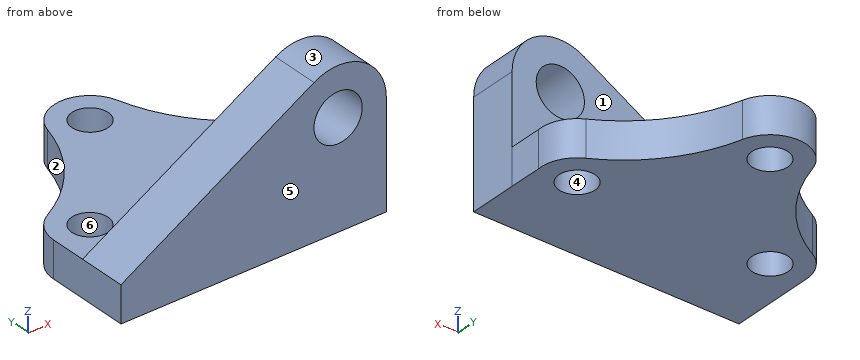
```python
from build123d import *

# Parameters (mm, degrees)
BASE_WEDGE_PROFILE_SKETCH_R     = 10
BASE_WEDGE_BLOCK_DEPTH          = 20
UPRIGHT_FLANGE_PROFILE_SKETCH_R = 7.5
UPRIGHT_FLANGE_PROFILE_SKETCH_W = 110
UPRIGHT_FLANGE_PROFILE_SKETCH_H = 20
UPRIGHT_FLANGE_WITH_HOLES_DEPTH = 15


with BuildPart() as part:
    # Base Wedge Profile Sketch → Base Wedge Block (new body)
    with BuildSketch(Plane(origin=(0, 0, 0), x_dir=(1, 0, 0), z_dir=(0, 1, 0))):
        with BuildLine():
            Line((0, 0), (110, 0))
            Line((110, 0), (110, -28.867513459))
            ThreePointArc((110, -28.867513459), (100, -46.188021535), (80, -46.188021535))
            Line((80, -46.188021535), (0, 0))
        make_face()
        with Locations(Location((90, -28.867513459, 0), (0, 0, 270))):
            Circle(BASE_WEDGE_PROFILE_SKETCH_R, mode=Mode.SUBTRACT)
    extrude(amount=-BASE_WEDGE_BLOCK_DEPTH)

    # Upright Flange Profile Sketch → Upright Flange with Holes (add)
    # profile 1 of 2: a face of its own
    with BuildSketch(Plane(origin=(0, 0, 0), x_dir=(-1, 0, 0), z_dir=(0, 0, -1))):
        with BuildLine():
            ThreePointArc((-40.373259229, 68.883899859), (-28.414925005, 45.194724357), (-7.985616598, 28.258899859))
            ThreePointArc((-7.985616598, 28.258899859), (-2.150569059, 22.739000225), (0, 15))
            Line((0, 15), (0, 0))
            Line((0, 0), (-110, 0))
            Line((-110, 0), (-109.941701745, 13.678807753))
            ThreePointArc((-109.941701745, 13.678807753), (-108.161756455, 22.195009869), (-101.953967939, 28.290685833))
            ThreePointArc((-101.953967939, 28.290685833), (-81.399813181, 45.193056262), (-69.341610571, 68.915685833))
            ThreePointArc((-69.341610571, 68.915685833), (-54.845255035, 79.99999097), (-40.373259229, 68.883899859))
        make_face()
        with Locations((-54.861714008, 65)):
            Circle(UPRIGHT_FLANGE_PROFILE_SKETCH_R, mode=Mode.SUBTRACT)
        with Locations((-15, 15)):
            Circle(UPRIGHT_FLANGE_PROFILE_SKETCH_R, mode=Mode.SUBTRACT)
        with Locations((-95, 15)):
            Circle(UPRIGHT_FLANGE_PROFILE_SKETCH_R, mode=Mode.SUBTRACT)
    # profile 2 of 2: a face of its own
    with BuildSketch(Plane(origin=(0, 0, 0), x_dir=(-1, 0, 0), z_dir=(0, 0, -1))):
        with Locations((-55, -10)):
            Rectangle(UPRIGHT_FLANGE_PROFILE_SKETCH_W, UPRIGHT_FLANGE_PROFILE_SKETCH_H)
    extrude(amount=UPRIGHT_FLANGE_WITH_HOLES_DEPTH)


solid = part.part
```
Design review of the part built by this model. Coordinates are the model's own, in mm. Face numbers are marked on the shaded views. A direction names the side the tool comes from. Coordinates: 2 decimals unless noted, no trailing zeros. Write each loop counter-clockwise with the first axis right and the second up, starting at its lowest first coordinate (ties: lowest second). Pieces come first, ordered by that corner, then holes.
1) To check wall thickness, follow L1, parallel to Z at x = 62.5, y = 6; L2, parallel to Y at x = 86, z = 0.5; L3, parallel to Z at x = 88, y = -8. State the ranges of each line that lie inside material, in increasing order.
2) Add section A-A (x = 90). Write out the cut boundary in (y, z), plus the area to 3 significant figures.
3) Machinability: for the marked faces 1 and 2, which of the approach directions +Z, -Z, +X, -X, +Y, -Y give a long, thin tool a straight path to every point of the face, cutting with its end or side? Answer none if there is none.
4) Add section D-D (z = 23.5). Write out the cut boundary in (x, y).
5) Add section B-B (z = -4). Write out the cut boundary in (x, y).
6) Mouldability with a two-part tool opening along Y and no side actions: class the marked faces 3, 4, 5 and 6 as +Y half, -Y half, draft (parallel to the pull), parting line (faces both ways), or undercut.
7) Insertion check: pin 1 (2 mm diameter, centred on x = 90.5, y = 36.5, fed in from +Z); pin 2 (9 mm diameter, centred on x = 15, y = 15, fed in from -Z); pin 3 (4 mm diameter, centred on x = 84, z = 39, fed in from +Y). Each pin has a flat end and moves straight along its axis. Give the tip position at first contact, or say it passes through.
8) Add section C-C (y = -4.5). Write out the cut boundary in (x, z).
Check result:
1. L1: z = -15 to 0
1. L2: y = -20 to 0
1. L3: z = -15 to 19.07, 38.67 to 48.77
2. outline: (-20, -15) - (9.41, -15) - (9.41, 0) - (0, 0) - (0, 18.87) - (-20, 18.87) - close; (-20, 38.87) - (0, 38.87) - (0, 48.87) - (-20, 48.87) - close; (20.59, -15) - (36.35, -15) - (36.35, 0) - (20.59, 0) - close
2. area: 1,250 mm2
3. face 1: +Z, +X, -X, +Y
3. face 2: +Z, -Z, -X, +Y
4. outline: (40.7, -20) - (81.56, -20) - (81.56, 0) - (40.7, 0) - close; (98.44, -20) - (110, -20) - (110, 0) - (98.44, 0) - close
5. outline: (0, -20) - (110, -20) - (110, 0) - (109.94, 13.68) arc R15 ccw to (101.95, 28.29) arc R65 cw to (69.34, 68.92) arc R15 ccw to (40.37, 68.88) arc R65 cw to (7.99, 28.26) arc R15 ccw to (0, 15) - close; hole circle Ø15 at (15, 15); hole circle Ø15 at (54.86, 65); hole circle Ø15 at (95, 15)
6. face 3: draft
6. face 4: undercut
6. face 5: -Y half
6. face 6: undercut
7. pin 1: stops at z = 0
7. pin 2: passes through
7. pin 3: stops at y = 0
8. outline: (0, -15) - (110, -15) - (110, 28.87) arc R20 ccw to (80, 46.19) - (0, 0) - close; hole circle Ø20 at (90, 28.87)
